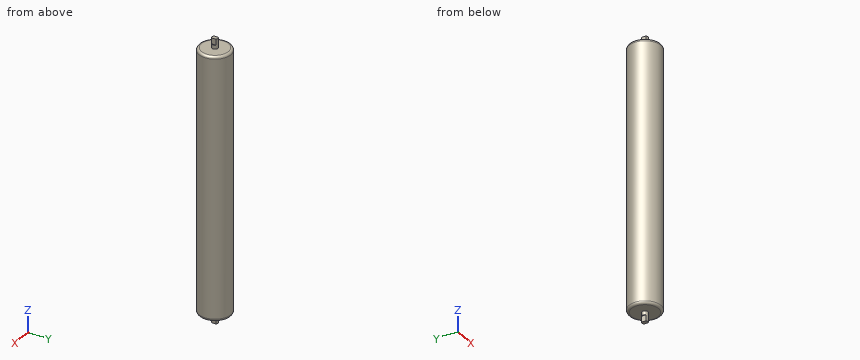
```python
from build123d import *

# Parameters (mm, degrees)
SKETCH_1_R           = 32.5
EXTRUDE_1_DEPTH      = 267.5
SKETCH_2_R           = 6
EXTRUDE_2_DEPTH      = 20
SKETCH_3_OUTSIDE_W   = 179.512
SKETCH_3_OUTSIDE_H   = 179.512
SKETCH_3_OUTSIDE_W_2 = 8
SKETCH_3_OUTSIDE_H_2 = 12.842917612
CUT_EXTRUDE_1_DEPTH  = 12
FILLET_1_R           = 5


with BuildPart() as part:
    # 草图1 → 凸台-拉伸1 (new, symmetric)
    with BuildSketch(Plane.XY):
        Circle(SKETCH_1_R)
    extrude(amount=EXTRUDE_1_DEPTH, both=True)

    # 草图2 → 凸台-拉伸2 (add)
    with BuildSketch(Plane(origin=(0, 0, -267.5), x_dir=(-1, 0, 0), z_dir=(0, 0, -1))):
        with Locations(Location((0, 0, 0), (0, 0, 180))):
            Circle(SKETCH_2_R)
    extrude_2 = extrude(amount=EXTRUDE_2_DEPTH)

    # 草图3 outside → 切除-拉伸1 (cut)
    with BuildSketch(Plane(origin=(0, 0, -287.5), x_dir=(-1, 0, 0), z_dir=(0, 0, -1))):
        Rectangle(SKETCH_3_OUTSIDE_W, SKETCH_3_OUTSIDE_H)
        Rectangle(SKETCH_3_OUTSIDE_W_2, SKETCH_3_OUTSIDE_H_2, mode=Mode.SUBTRACT)
    cut_extrude_1 = extrude(amount=-CUT_EXTRUDE_1_DEPTH, mode=Mode.SUBTRACT)

    # 镜向1: 凸台-拉伸2, 切除-拉伸1 across plane
    add(extrude_2.mirror(Plane.XY))
    add(cut_extrude_1.mirror(Plane.XY), mode=Mode.SUBTRACT)

    # 圆角1
    fillet_1_edges = [part.edges().sort_by_distance(p)[0] for p in [
        (-32.5, 0, -267.5),
        (-32.5, 0, 267.5),
    ]]
    fillet(fillet_1_edges, radius=FILLET_1_R)


solid = part.part
```
Part model, mm, in its own coordinate system. Give positions to 0.01 mm unless a question says otherwise; leave off trailing zeros. Write each loop counter-clockwise with the first axis right and the second up, starting at its lowest first coordinate (ties: lowest second). Pieces come first, ordered by that corner, then holes. Notation, with made-up numbers: (26.5, 34) -> (59.5, 34) arc R21 ccw to (59.5, 64) -> close; hole circle Ø5 at (47.25, 64.25). An arc over 180 degrees is marked (long way). Put each result on its own line as item: value. Start each with the question number.
Item 1: Pin check, flat tips, straight feed: pin 1 Ø3 at (x, y) = (-2.5, -18) entering from +Z; pin 2 Ø1.6 at (x, y) = (-5, 1.5) entering from +Z; pin 3 Ø8 at (y, z) = (6, 224.5) entering from +X; pin 4 Ø16.5 at (x, y) = (7, 9) entering from +Z. Stop position of each tip, or through.
Item 2: Cut at A-A (z = -179). List the corners of the cut face in (x, y).
Item 3: Wall check: L1, parallel to Z at x = -4.5, y = 19; L2, parallel to X at y = 2, z = -99; L3, parallel to X at y = -28, z = -224. Give the ranges that are in metal, low to high. Write a range as [from, to].
Answer list:
1. pin 1: stops at z = 267.5
1. pin 2: stops at z = 275.5
1. pin 3: stops at x = 32.44
1. pin 4: stops at z = 287.5
2. outline: circle Ø65 at (0, 0)
3. L1: z = [-267.5, 267.5]
3. L2: x = [-32.44, 32.44]
3. L3: x = [-16.5, 16.5]
